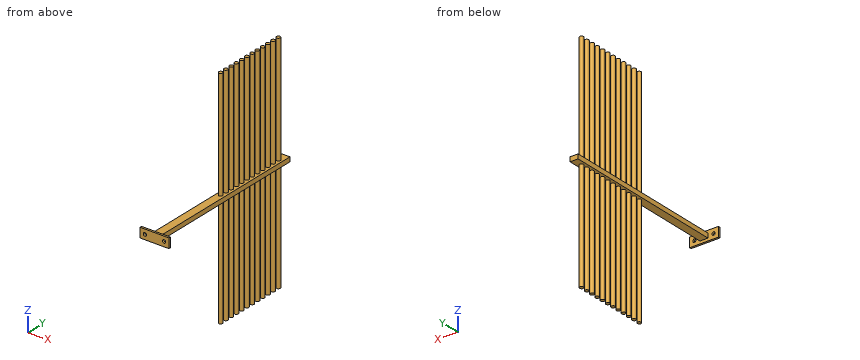
from build123d import *

# Parameters (mm, degrees)
SKETCH1_W                = 25
SKETCH1_H                = 520
BOSS_EXTRUDE1_DEPTH      = 14
BOSS_EXTRUDE2_START      = -7
SKETCH3_R                = 6
BOSS_EXTRUDE2_DEPTH      = 350
LPATTERN1_COUNT          = 12
LPATTERN1_PITCH          = 21
SKETCH4_W                = 90
SKETCH4_H                = 30
BOSS_EXTRUDE3_DEPTH      = 6
M8_CLEARANCE_HOLE1_D     = 10
M8_CLEARANCE_HOLE1_DEPTH = 20
M8_CLEARANCE_HOLE1_TIP   = 3.004303095


with BuildPart() as part:
    # Sketch1 → Boss-Extrude1 (new body)
    with BuildSketch(Plane.XY):
        Rectangle(SKETCH1_W, SKETCH1_H)
    extrude(amount=BOSS_EXTRUDE1_DEPTH)

    # Sketch3 → Boss-Extrude2 (add, symmetric)
    with BuildSketch(Plane.XY.offset(14).offset(BOSS_EXTRUDE2_START)):
        with Locations((0, 230)):
            Circle(SKETCH3_R)
    boss_extrude2 = extrude(amount=BOSS_EXTRUDE2_DEPTH, both=True)

    # LPattern1: Boss-Extrude2 ×12
    with Locations(*[(0, -i * LPATTERN1_PITCH, 0) for i in range(1, LPATTERN1_COUNT)]):
        add(boss_extrude2)

    # Sketch4 → Boss-Extrude3 (add)
    with BuildSketch(Plane.XZ.offset(260)):
        with Locations((0, 7)):
            Rectangle(SKETCH4_W, SKETCH4_H)
    extrude(amount=BOSS_EXTRUDE3_DEPTH)

    # M8 Clearance Hole1
    with Locations(Plane(origin=(0, -260, 0), x_dir=(1, 0, 0), z_dir=(0, 1, 0))):
        with Locations((-30, -7), (30, -7)):
            Hole(M8_CLEARANCE_HOLE1_D / 2, depth=M8_CLEARANCE_HOLE1_DEPTH)
            with Locations((0, 0, -(M8_CLEARANCE_HOLE1_DEPTH + M8_CLEARANCE_HOLE1_TIP / 2))):  # 118° drill point
                Cone(0, M8_CLEARANCE_HOLE1_D / 2, M8_CLEARANCE_HOLE1_TIP, mode=Mode.SUBTRACT)


solid = part.part
The listing builds one solid part. Answer for the finished solid, in the listing's coordinates (mm). Give positions to 0.01 mm unless a question says otherwise; leave off trailing zeros. Order: outer loops, then holes, each group sorted by start corner. A loop starts at its lowest first (then second) coordinate and runs counter-clockwise, first axis right, second up. Notation, with made-up numbers: (48.5, 15) -> (70.5, 15) arc R20 ccw to (70.5, 41) -> close; hole circle Ø5 at (-26, 85.5). An arc over 180 degrees is marked (long way). Put each result on its own line as item: value.
Item 1: Given P1, Ø11, axis at y = 14, z = 5, coming from the -X side; P2, Ø12.5, axis at x = 1.5, y = -58, coming from the +Z side; P3, Ø4, axis at y = 174.5, z = -216, coming from the +X side; P4, Ø15, axis at x = 16.5, z = 7, coming from the +Y side, each flat-ended and moving along its own axis, determine where each tip first touches the part or whether it passes through.
Established:
P1: stops at x = -12.5
P2: stops at z = 14
P3: stops at x = 2.4
P4: stops at y = 260
Item 2: A cutting plane is placed at B-B on y = -79.5. Give the vertices of the cut face in (x, z), plus the area to 3 significant figures.
Established:
outline: (-12.5, 0) -> (12.5, 0) -> (12.5, 14) -> (-12.5, 14) -> close
area: 350 mm^2
Item 3: A cutting plane is placed at A-A on z = 289.5. Count the separate pieces of the cut face and the enclosed holes in it, plus the area to 3 significant figures.
Established:
separate pieces: 12
enclosed holes: 0
area: 1,360 mm^2
Item 4: Straight lines are drawn through the part: line 1 (Z direction, x = 30, y = -264); line 2 (Z direction, x = 2, y = -224.5); line 3 (X direction, y = 103, z = -39). For each, find the intervals that lie inside material, in ascending order.
Established:
line 1: z = -8 to 2, 12 to 22
line 2: z = 0 to 14
line 3: x = -5.92 to 5.92
